Read the model definition and answer for the solid it produces. Units are mm, in the model's axes. Round coordinates to 2 decimals unless told otherwise and drop trailing zeros. Order: outer loops, then holes, each group sorted by start corner. A loop starts at its lowest first (then second) coordinate and runs counter-clockwise, first axis right, second up. Notation, with made-up numbers: (31, 24) -> (44, 24) arc R10 cw to (44, 29) -> close; hole circle Ø4 at (64.5, 44). An arc over 180 degrees is marked (long way). Answer as a JSON object with one key per item and string values. Group by question number.
Item 1: Section A-A, the plane x = 166.5 is taken. Write down the section's boundary in (y, z).
Item 2: Consider probe 1 along Z at (x, y) = (-259, -2); probe 2 along X at (y, z) = (-16, -2); probe 3 along Y at (x, z) = (-540, -6). Determine where each line is inside the solid, lowest interval first. Write a range as from..to.
Item 3: Given P1, Ø8, axis at x = 155, y = 10.5, coming from the -Z side; P2, Ø1.7, axis at x = 727, y = 13, coming from the +Z side; P3, Ø3, axis at x = 130.5, z = -15.5, coming from the -Y side, each flat-ended and moving along its own axis, determine where each tip first touches the part or whether it passes through.
from build123d import *

# Parameters (mm, degrees)
CUT_EXTRUDE1_DEPTH = 4
CHAMFER1_SIZE      = 1


with BuildPart() as part:
    # Sketch1 → Revolve1 (revolve)
    with BuildSketch(Plane.XY, mode=Mode.PRIVATE) as revolve1_sk:
        Polygon((-738, 15), (-700, 15), (-700, 20), (700, 20), (700, 15), (738, 15), (738, 0), (-738, 0), align=None)
    revolve(revolve1_sk.sketch.rotate(Axis((738, 0, 0), (-1, 0, 0)), 90), axis=Axis((738, 0, 0), (-1, 0, 0)))

    # Sketch3 → Cut-Extrude1 (cut)
    with BuildSketch(Plane(origin=(0, 15, 0), x_dir=(1, 0, 0), z_dir=(0, 1, 0))):
        with BuildLine():
            Line((-705, 4), (-738, 4))
            Line((-738, 4), (-738, -4))
            Line((-738, -4), (-705, -4))
            ThreePointArc((-705, -4), (-701, 0), (-705, 4))
        make_face()
    cut_extrude1 = extrude(amount=-CUT_EXTRUDE1_DEPTH, mode=Mode.SUBTRACT)

    # Mirror1: Cut-Extrude1 across plane
    add(cut_extrude1.mirror(Plane.ZY), mode=Mode.SUBTRACT)

    # Chamfer1
    chamfer1_edges = [part.edges().sort_by_distance(p)[0] for p in [
        (-738, -11.937336386, 9.082951062),
        (738, -11.937336386, 9.082951062),
        (700, 0, 20),
        (-700, 0, 20),
    ]]
    chamfer(chamfer1_edges, length=CHAMFER1_SIZE)


solid = part.part
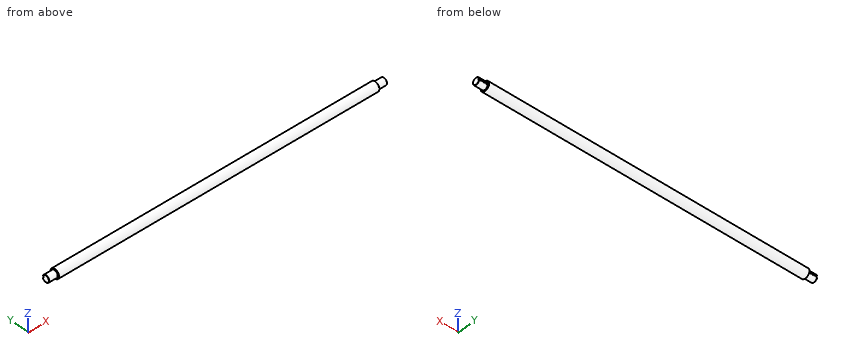
Values found:
{
 "1": {"outline": "circle Ø40 at (0, 0)"},
 "2": {"probe 1": "-19.9..19.9", "probe 2": "-700..700", "probe 3": "-19.08..19.08"},
 "3": {"P1": "z = -18.91", "P2": "z = 8.8", "P3": "y = -14.28"}
}
